The listing builds one solid part. Answer for the finished solid, in the listing's coordinates (mm). A direction names the side the tool comes from. Round coordinates to 2 decimals unless told otherwise and drop trailing zeros. Loops run counter-clockwise (first coordinate to the right, second up) from the corner with the lowest first, then second, coordinate; pieces in that order, holes last. Notation, with made-up numbers: (5, -14.5) - (47, -14.5) arc R24 ccw to (47, 16.5) - close; hole circle Ø10 at (-21, -31). An arc over 180 degrees is marked (long way). Write item = value, one per line. Start each with the question number.
1) Given pin 1 Ø6 at (x, z) = (50, 28) entering from +Y; pin 2 Ø17 at (x, y) = (0, 67) entering from -Z; pin 3 Ø12 at (x, z) = (55, 50) entering from +Y; pin 4 Ø8.5 at (x, y) = (47.38, 47.38) entering from +Z, each flat-ended and moving along its own axis, determine where each tip first touches the part or whether it passes through.
2) A tool of negligible diameter and unlimited length cuts with its end or side. For faces 1 (the flat face through (-23.5, 52.4, 9)), 2 (the cylindrical face through (-47.69, 15.02, 29.58)), 3 (the cylindrical face through (-48.067, -42.147, 4.437)), from which of +Z, -Z, +X, -X, +Y, -Y can it reach the whole face along a straight path? Write none if from no direction.
3) Straight lines are drawn through the part: line 1 along X through (y, z) = (52, 7); line 2 along Z through (x, y) = (-66.5, -11); line 3 along X through (y, z) = (1.5, 56). For each, find the intervals that lie inside material, in ascending order.
4) Section A-A, the plane x = 0 is taken. Give the number of separate pieces and of enclosed holes in the cut face, and give its area (3 significant figures).
5) Section D-D, the plane x = 67 is taken. Determine the outline of the cut face in (y, z) (3 decimals).
6) For a pull along X with two mould halves and no side action, classify faces 4 (the flat face through (-22, -41, 60)), 5 (the cylindrical face through (-11.923, -53.692, 36.636)), 6 (the flat face through (-1, -51, 0)) as released by +X, released by -X, zero draft, split by the parting line, or undercut.
7) Section B-B, the plane y = 64.5 is taken. Determine the outline of the cut face in (x, z).
from build123d import *

# Parameters (mm, degrees)
SKETCH1_R           = 78
BOSS_EXTRUDE1_DEPTH = 9
SKETCH2_R           = 55
BOSS_EXTRUDE2_DEPTH = 56
SKETCH3_R           = 50
CUT_EXTRUDE2_DEPTH  = 60
SKETCH4_R           = 46
CUT_EXTRUDE3_DEPTH  = 129.035151423
SKETCH5_R           = 5.275
CUT_EXTRUDE4_DEPTH  = 129.035151423
CIRPATTERN1_COUNT   = 8
CHAMFER1_SIZE       = 2
FILLET1_R           = 2


with BuildPart() as part:
    # Sketch1 → Boss-Extrude1 (new body)
    with BuildSketch(Plane.XY):
        Circle(SKETCH1_R)
    extrude(amount=BOSS_EXTRUDE1_DEPTH)

    # Sketch2 → Boss-Extrude2 (add)
    with BuildSketch(Plane.XY.offset(9)):
        Circle(SKETCH2_R)
    extrude(amount=BOSS_EXTRUDE2_DEPTH)

    # Sketch3 → Cut-Extrude2 (cut)
    with BuildSketch(Plane(origin=(0, 0, 0), x_dir=(-1, 0, 0), z_dir=(0, 0, -1))):
        Circle(SKETCH3_R)
    extrude(amount=-CUT_EXTRUDE2_DEPTH, mode=Mode.SUBTRACT)

    # Sketch4 → Cut-Extrude3 (cut, through all)
    with BuildSketch(Plane.XY.offset(65)):
        Circle(SKETCH4_R)
    extrude(amount=-CUT_EXTRUDE3_DEPTH, mode=Mode.SUBTRACT)

    # Sketch5 → Cut-Extrude4 (cut, through all)
    with BuildSketch(Plane(origin=(0, 0, 0), x_dir=(-1, 0, 0), z_dir=(0, 0, -1))):
        with Locations((0, 67)):
            Circle(SKETCH5_R)
    cut_extrude4 = extrude(amount=-CUT_EXTRUDE4_DEPTH, mode=Mode.SUBTRACT)

    # CirPattern1: Cut-Extrude4 ×8 about axis
    cirpattern1_axis = Axis((0, 0, 0), (0, 0, 1))
    for i in range(1, CIRPATTERN1_COUNT):
        add(cut_extrude4.rotate(cirpattern1_axis, i * 360 / CIRPATTERN1_COUNT), mode=Mode.SUBTRACT)

    # Chamfer1
    chamfer1_edges = [part.edges().sort_by_distance(p)[0] for p in [
        (-46, 0, 65),
        (-55, 0, 65),
    ]]
    chamfer(chamfer1_edges, length=CHAMFER1_SIZE)

    # Fillet1
    fillet1_edges = [part.edges().sort_by_distance(p)[0] for p in [
        (-55, 0, 9),
    ]]
    fillet(fillet1_edges, radius=FILLET1_R)


solid = part.part
Geometry check:
q1.pin_1 = 28.57
q1.pin_2 = 0
q1.pin_3 = 24.98
q1.pin_4 = through
q2.face_1 = +Z
q2.face_2 = -Z
q2.face_3 = +Z, -Z
q3.line_1 = -58.14 to -49.91, -44.84 to 44.84, 49.91 to 58.14
q3.line_2 = 0 to 9
q3.line_3 = -54.98 to -49.98, 49.98 to 54.98
q4.separate_pieces = 4
q4.enclosed_holes = 0
q4.area = 908 mm2
q5.outline = (-39.937, 0) - (-5.275, 0) - (-5.275, 9) - (-39.937, 9) - close; (5.275, 0) - (39.937, 0) - (39.937, 9) - (5.275, 9) - close
q6.face_4 = undercut
q6.face_5 = split by the parting line
q6.face_6 = zero draft
q7.outline = (-43.86, 0) - (-4.64, 0) - (-4.64, 9) - (-43.86, 9) - close; (4.64, 0) - (43.86, 0) - (43.86, 9) - (4.64, 9) - close
